Model file for the job. Use its own axes, mm. A direction names the side the tool comes from. Round coordinates to 2 decimals unless told otherwise and drop trailing zeros. Order: outer loops, then holes, each group sorted by start corner. A loop starts at its lowest first (then second) coordinate and runs counter-clockwise, first axis right, second up. Notation, with made-up numbers: M 28,48 L 74,48 A19 cw 74,57 Z; hole C -26,-4 d4. An arc over 180 degrees is marked long. Return JSON: item names as keys, results as strings. Group by question number.
Item 1: Slice it at A-A on x = -54. Write the cut outline in (y, z), then the cut area to 3 significant figures.
Item 2: Slice it at C-C on z = 124. Write the cut outline in (x, y).
Item 3: Pull direction Y, two halves, no side cores. Call faces 1 (the face through (-1, 1, 0)), 2 (the face through (-51.42, 56.365, 139.86)), 3 (the face through (-44, -63, 66)): pulls with the +Y half, pulls with the -Y half, needs draft (parallel to the pull), parting line crosses it, or undercut.
Item 4: Probe line 1 along Y through (x, z) = (-54, 143.25); line 2 along Y through (x, z) = (-54.5, 95). List the from-to ranges inside material, lowest first.
Item 5: Pin check, flat tips, straight feed: pin 1 Ø3 at (y, z) = (53, 60.5) entering from -X; pin 2 Ø3 at (y, z) = (-56, 33.5) entering from +X; pin 3 Ø7.5 at (x, y) = (50.5, -52.5) entering from -Z; pin 4 Ø20 at (x, y) = (53, 55) entering from -Z. Stop position of each tip, or through.
Item 6: Which spindle directions (+Z, -Z, +X, -X, +Y, -Y) get a long thin tool onto all of the face, cutting with end or side? Do faces 4 (the face through (-50, -53, 130)), 5 (the face through (47, -46, 66)), 6 (the face through (-53, 50, 130)). Say none if no direction does.
from build123d import *

# Parameters (mm, degrees)
SKETCH1_W           = 130
SKETCH1_H           = 130
BOSS_EXTRUDE1_DEPTH = 150
FILLET1_R           = 20
SKETCH2_W           = 69.063294878
SKETCH2_H           = 85.712482036
CUT_EXTRUDE1_DEPTH  = 130
CIRPATTERN1_COUNT   = 4
FILLET2_R           = 5
FILLET3_R           = 5
SKETCH4_R           = 3.5
CUT_EXTRUDE2_DEPTH  = 40
CIRPATTERN2_COUNT   = 4


with BuildPart() as part:
    # Sketch1 → Boss-Extrude1 (new body)
    with BuildSketch(Plane.XY):
        Rectangle(SKETCH1_W, SKETCH1_H)
    extrude(amount=BOSS_EXTRUDE1_DEPTH)

    # Fillet1
    fillet1_edges = [part.edges().sort_by_distance(p)[0] for p in [
        (65, -65, 75),
        (-65, -65, 75),
        (-65, 65, 75),
        (65, 65, 75),
    ]]
    fillet(fillet1_edges, radius=FILLET1_R)

    # Sketch2 → Cut-Extrude1 (cut)
    with BuildSketch(Plane(origin=(0, 0, 0), x_dir=(-1, 0, 0), z_dir=(0, 0, -1))):
        with Locations((-79.531647439, 87.856241018)):
            Rectangle(SKETCH2_W, SKETCH2_H)
    cut_extrude1 = extrude(amount=-CUT_EXTRUDE1_DEPTH, mode=Mode.SUBTRACT)

    # CirPattern1: Cut-Extrude1 ×4 about axis
    cirpattern1_axis = Axis((0, 0, 0), (0, 0, 1))
    for i in range(1, CIRPATTERN1_COUNT):
        add(cut_extrude1.rotate(cirpattern1_axis, i * 360 / CIRPATTERN1_COUNT), mode=Mode.SUBTRACT)

    # Fillet2
    fillet2_edges = [part.edges().sort_by_distance(p)[0] for p in [
        (45, 45, 65),
        (-45, 45, 65),
        (-45, -45, 65),
        (45, -45, 65),
    ]]
    fillet(fillet2_edges, radius=FILLET2_R)

    # Fillet3
    fillet3_edges = [part.edges().sort_by_distance(p)[0] for p in [
        (45, -65, 65),
        (-65, -45, 65),
        (65, 45, 65),
        (-45, 65, 65),
        (45, 65, 65),
        (-65, 45, 65),
        (65, -45, 65),
        (-45, -65, 65),
    ]]
    fillet(fillet3_edges, radius=FILLET3_R)

    # Sketch4 → Cut-Extrude2 (cut)
    with BuildSketch(Plane(origin=(0, 0, 130), x_dir=(-1, 0, 0), z_dir=(0, 0, -1))):
        with Locations((54, 54)):
            Circle(SKETCH4_R)
    cut_extrude2 = extrude(amount=-CUT_EXTRUDE2_DEPTH, mode=Mode.SUBTRACT)

    # CirPattern2: Cut-Extrude2 ×4 about axis
    cirpattern2_axis = Axis((0, 0, 0), (0, 0, 1))
    for i in range(1, CIRPATTERN2_COUNT):
        add(cut_extrude2.rotate(cirpattern2_axis, i * 360 / CIRPATTERN2_COUNT), mode=Mode.SUBTRACT)


solid = part.part
Output values:
{
 "1": {"outline": "M -62.86,130 L -57.5,130 L -57.5,150 L -62.86,150 Z; M -50.5,130 L -45,130 L -45,0 L 45,0 L 45,130 L 50.5,130 L 50.5,150 L -50.5,150 Z; M 57.5,130 L 62.86,130 L 62.86,150 L 57.5,150 Z", "area": "13,900 mm²"},
 "2": {"outline": "M -65,-40 A5 ccw -60,-45 L -50,-45 A5 cw -45,-50 L -45,-60 A5 ccw -40,-65 L 40,-65 A5 ccw 45,-60 L 45,-50 A5 cw 50,-45 L 60,-45 A5 ccw 65,-40 L 65,40 A5 ccw 60,45 L 50,45 A5 cw 45,50 L 45,60 A5 ccw 40,65 L -40,65 A5 ccw -45,60 L -45,50 A5 cw -50,45 L -60,45 A5 ccw -65,40 Z"},
 "3": {"face 1": "needs draft", "face 2": "undercut", "face 3": "pulls with the -Y half"},
 "4": {"line 1": "-62.86 to -57.5, -50.5 to 50.5, 57.5 to 62.86", "line 2": "-45 to 45"},
 "5": {"pin 1": "x = -45", "pin 2": "x = 45", "pin 3": "z = 130", "pin 4": "z = 0"},
 "6": {"face 4": "-Z, -X, -Y", "face 5": "-Z, +X, -Y", "face 6": "-Z, -X, +Y"}
}
